Part model, mm, in its own coordinate system. Face numbers are marked on the shaded views. Give positions to 0.01 mm unless a question says otherwise; leave off trailing zeros. Order: outer loops, then holes, each group sorted by start corner. A loop starts at its lowest first (then second) coordinate and runs counter-clockwise, first axis right, second up. Notation, with made-up numbers: (80.5, 88) -> (125.5, 88) arc R36 ccw to (125.5, 126) -> close; hole circle Ø3 at (12.25, -28). An arc over 180 degrees is marked (long way). Write item = value, one per line. Start each with the question number.
Item 1: Band-saw the part on B-B on x = -52.5. Write the cut outline in (y, z), plus the area to 3 significant figures.
Item 2: Band-saw the part on A-A on y = 0. Write the cut outline in (x, z), plus the area to 3 significant figures.
Item 3: Band-saw the part on C-C on z = 1592.5. Write the cut outline in (x, y).
Item 4: Flat gauge pins, fed straight in: P1, Ø13, axis at x = 121.5, z = 333, coming from the -Y side; P2, Ø3.5, axis at x = 119.5, z = 347, coming from the +Y side. Where does each tip first touch, or does it go through?
Item 5: Drill centre lines: line 1 along Y through (x, z) = (-50, 1008); line 2 along Y through (x, z) = (108.5, 1148). Where is each one in solid material? Low to high.
Item 6: Pull direction Y, two halves, no side cores. Call the marked faces 1, 2, 3 and 4: +Y half, -Y half, draft (parallel to the pull), parting line (faces both ways), or undercut.
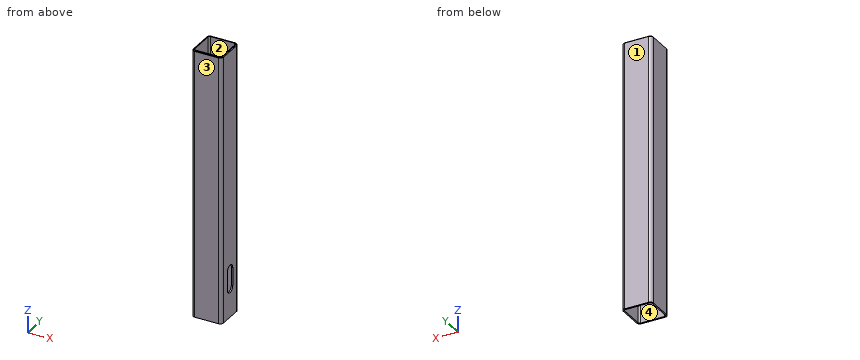
```python
from build123d import *

# Parameters (mm, degrees)
EXTRUDE_1_DEPTH     = 2220
CHAMFER_1_SIZE      = 5
CUT_EXTRUDE_1_REACH = 2239.527


with BuildPart() as part:
    # 草图1 → 凸台-拉伸1 (new body)
    with BuildSketch(Plane.XY):
        with BuildLine():
            Line((-99, 125), (99, 125))
            ThreePointArc((99, 125), (117.384776311, 117.384776311), (125, 99))
            Line((125, 99), (125, -99))
            ThreePointArc((125, -99), (117.384776311, -117.384776311), (99, -125))
            Line((99, -125), (-99, -125))
            ThreePointArc((-99, -125), (-117.384776311, -117.384776311), (-125, -99))
            Line((-125, -99), (-125, 99))
            ThreePointArc((-125, 99), (-117.384776311, 117.384776311), (-99, 125))
        make_face()
        with BuildLine():
            Line((-99, 113), (99, 113))
            ThreePointArc((99, 113), (108.899494937, 108.899494937), (113, 99))
            Line((113, 99), (113, -99))
            ThreePointArc((113, -99), (108.899494937, -108.899494937), (99, -113))
            Line((99, -113), (-99, -113))
            ThreePointArc((-99, -113), (-108.899494937, -108.899494937), (-113, -99))
            Line((-113, -99), (-113, 99))
            ThreePointArc((-113, 99), (-108.899494937, 108.899494937), (-99, 113))
        make_face(mode=Mode.SUBTRACT)
    extrude(amount=EXTRUDE_1_DEPTH)

    # 倒角1
    chamfer_1_edges = [part.edges().sort_by_distance(p)[0] for p in [
        (-117.384776311, -117.384776311, 2220),
        (0, -125, 2220),
        (117.384776311, -117.384776311, 2220),
        (125, 0, 2220),
        (117.384776311, 117.384776311, 2220),
        (0, 125, 2220),
        (-117.384776311, 117.384776311, 2220),
        (-125, 0, 2220),
    ]]
    chamfer(chamfer_1_edges, length=CHAMFER_1_SIZE)

    # 草图2 → 切除-拉伸1 (cut, up to next)
    with BuildSketch(Plane(origin=(125, 0, 0), x_dir=(0, 0, -1), z_dir=(1, 0, 0)), mode=Mode.PRIVATE) as cut_extrude_1_sk1:
        with BuildLine():
            Line((-395, 40), (-245, 40))
            ThreePointArc((-245, 40), (-205, 0), (-245, -40))
            Line((-245, -40), (-395, -40))
            ThreePointArc((-395, -40), (-435, 0), (-395, 40))
        make_face()
    cut_extrude_1_tool1 = extrude(cut_extrude_1_sk1.sketch, amount=-CUT_EXTRUDE_1_REACH, mode=Mode.PRIVATE) & part.part
    add(cut_extrude_1_tool1.solids().sort_by_distance((125, 0, 320))[0], mode=Mode.SUBTRACT)


solid = part.part
```
Values found:
q1.outline = (-125, 0) -> (-113, 0) -> (-113, 2220) -> (-120, 2220) -> (-125, 2215) -> close; (113, 0) -> (125, 0) -> (125, 2215) -> (120, 2220) -> (113, 2220) -> close
q1.area = 53,300 mm^2
q2.outline = (-125, 0) -> (-113, 0) -> (-113, 2220) -> (-120, 2220) -> (-125, 2215) -> close; (113, 0) -> (125, 0) -> (125, 205) -> (113, 205) -> close; (113, 435) -> (125, 435) -> (125, 2215) -> (120, 2220) -> (113, 2220) -> close
q2.area = 50,500 mm^2
q3.outline = (-125, -99) arc R26 ccw to (-99, -125) -> (99, -125) arc R26 ccw to (125, -99) -> (125, 99) arc R26 ccw to (99, 125) -> (-99, 125) arc R26 ccw to (-125, 99) -> close; hole (-113, -99) arc R14 ccw to (-99, -113) -> (99, -113) arc R14 ccw to (113, -99) -> (113, 99) arc R14 ccw to (99, 113) -> (-99, 113) arc R14 ccw to (-113, 99) -> close
q4.P1 = -119.49
q4.P2 = 117.01
q5.line_1 = -125 to -113, 113 to 125
q5.line_2 = -123.2 to -109.28, 109.28 to 123.2
q6.face_1 = +Y half
q6.face_2 = undercut
q6.face_3 = -Y half
q6.face_4 = undercut
